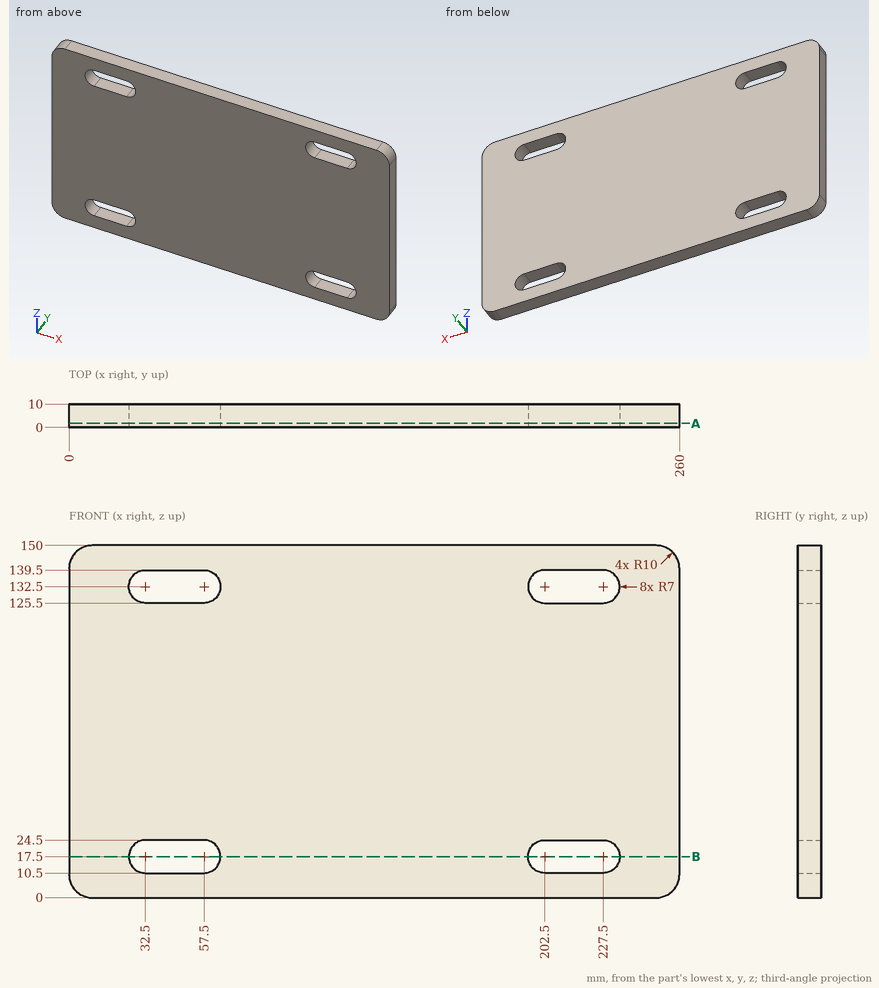
Part print with two shaded views. Sizes in mm from the minimum x, y, z corner. Round coordinates to 2 decimals unless told otherwise and drop trailing zeros. Loops run counter-clockwise (first coordinate to the right, second up) from the corner with the lowest first, then second, coordinate; pieces in that order, holes last. Notation, with made-up numbers: M 37,-6.75 L 57,-6.75 A21 ccw 57,5.25 Z; hole C -6,0.25 d11. An arc over 180 degrees is marked long. Return JSON: item names as keys, results as strings. Group by question number.
(1) Wall check: probe 1 along Z at (x, y) = (44.5, 2.5); probe 2 along Z at (x, y) = (27.5, 1); probe 3 along X at (y, z) = (9, 127). Give the ranges that are in metal, low to high. Write a range as [from, to].
(2) Saw through at B-B, the plane z = 17.5. List the corners of the cut face in (x, y), and give its area (3 significant figures).
(3) Saw through at A-A, the plane y = 1.75. List the corners of the cut face in (x, z).
(4) Drop a flat-ended pin along its axis: P1, Ø8, axis at x = 198.5, z = 16, coming from the +Y side. Give the stop position or say it passes through.
Answer list:
{
 "1": {"probe 1": "[0, 10.5], [24.5, 125.5], [139.5, 150]", "probe 2": "[0, 12.6], [22.4, 127.6], [137.4, 150]", "probe 3": "[0, 28.17], [61.83, 198.17], [231.83, 260]"},
 "2": {"outline": "M 0,0 L 25.5,0 L 25.5,10 L 0,10 Z; M 64.5,0 L 195.5,0 L 195.5,10 L 64.5,10 Z; M 234.5,0 L 260,0 L 260,10 L 234.5,10 Z", "area": "1,820 mm2"},
 "3": {"outline": "M 0,10 A10 ccw 10,0 L 250,0 A10 ccw 260,10 L 260,140 A10 ccw 250,150 L 10,150 A10 ccw 0,140 Z; hole M 32.5,10.5 L 57.5,10.5 A7 ccw 57.5,24.5 L 32.5,24.5 A7 ccw Z; hole M 32.5,125.5 L 57.5,125.5 A7 ccw 57.5,139.5 L 32.5,139.5 A7 ccw Z; hole M 202.5,10.5 L 227.5,10.5 A7 ccw 227.5,24.5 L 202.5,24.5 A7 ccw Z; hole M 202.5,125.5 L 227.5,125.5 A7 ccw 227.5,139.5 L 202.5,139.5 A7 ccw Z"},
 "4": {"P1": "y = 10"}
}
